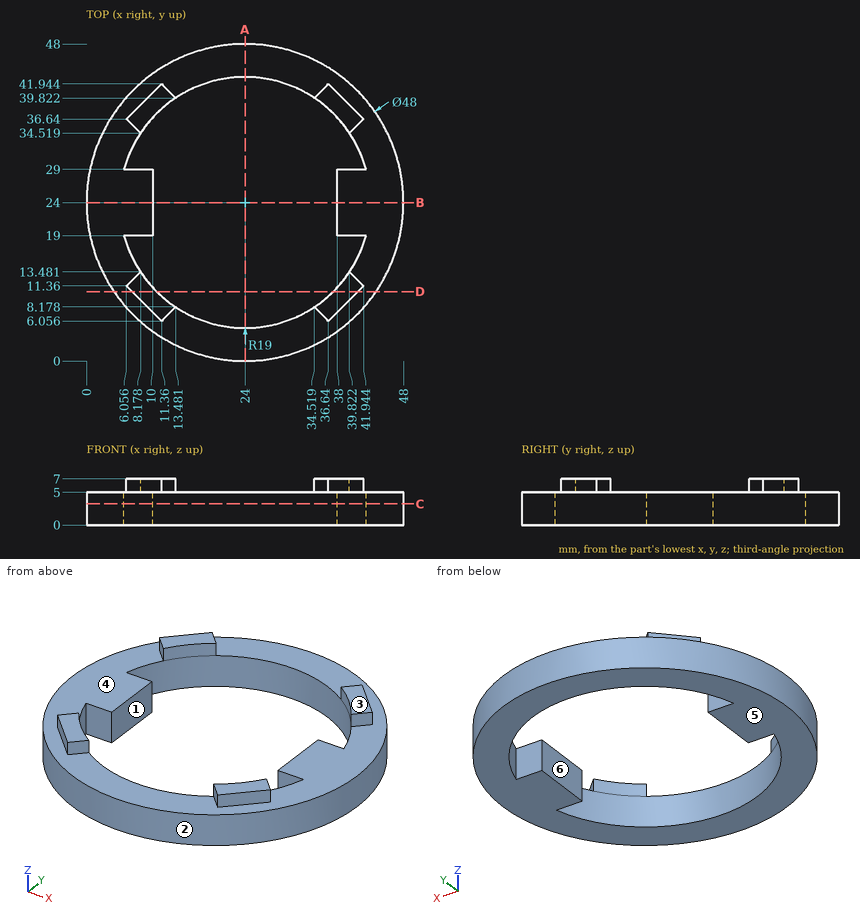
Part print with two shaded views. Sizes in mm from the minimum x, y, z corner. A direction names the side the tool comes from. Round coordinates to 2 decimals unless told otherwise and drop trailing zeros. Loops run counter-clockwise (first coordinate to the right, second up) from the corner with the lowest first, then second, coordinate; pieces in that order, holes last.
Item 1: Saw through at B-B (y = 24). List the corners of the cut face in (x, z).
Item 2: Which spindle directions (+Z, -Z, +X, -X, +Y, -Y) get a long thin tool onto all of the face, cutting with end or side? Do the marked faces 4, 5 and 6. Say none if no direction does.
Item 3: Two-plate mould, pull along Y, no slides. Class the marked faces 1, 2 and 3: released by +Y, released by -Y, zero draft, split by the parting line, or undercut.
Item 4: Saw through at D-D (y = 10.5). List the corners of the cut face in (x, z) (1 decimal).
Item 5: Saw through at A-A (x = 24). List the corners of the cut face in (y, z).
Item 6: Pin check, flat tips, straight feed: P1, Ø2, axis at y = 28, z = 3, coming from the -X side; P2, Ø4, axis at x = 33.5, z = 6, coming from the -Y side; P3, Ø3.5, axis at x = 39.5, z = 1.5, coming from the -Y side; P4, Ø6, axis at x = 17, y = 37.5, coming from the +Z side. Stop position of each tip, or through.
Item 7: Drill centre lines: line 1 along Y through (x, z) = (24.5, 3.25) (1 decimal); line 2 along Y through (x, z) = (7, 2.75) (1 decimal); line 3 along Z through (x, y) = (43, 16). Where is each one in solid material? Low to high.
Item 8: Saw through at C-C (z = 3.25). List the corners of the cut face in (x, y), then the cut area to 3 significant figures.
Worked answers:
1. outline: (0, 0) - (10, 0) - (10, 5) - (0, 5) - close; (38, 0) - (48, 0) - (48, 5) - (38, 5) - close
2. face 4: +Z
2. face 5: -Z, +X, -X, +Y, -Y
2. face 6: +Z, -Z
3. face 1: undercut
3. face 2: split by the parting line
3. face 3: zero draft
4. outline: (4.2, 0) - (10.6, 0) - (10.6, 7) - (6.9, 7) - (6.9, 5) - (4.2, 5) - close; (37.4, 0) - (43.8, 0) - (43.8, 5) - (41.1, 5) - (41.1, 7) - (37.4, 7) - close
5. outline: (0, 0) - (5, 0) - (5, 5) - (0, 5) - close; (43, 0) - (48, 0) - (48, 5) - (43, 5) - close
6. P1: stops at x = 0.19
6. P2: stops at y = 1.29
6. P3: stops at y = 4.33
6. P4: passes through
7. line 1: y = 0 to 5, 43 to 48
7. line 2: y = 7.1 to 15.5, 19 to 29, 32.5 to 40.9
7. line 3: z = 0 to 5
8. outline: circle Ø48 at (24, 24); hole (5.67, 19) arc R19 ccw to (42.33, 19) - (38, 19) - (38, 29) - (42.33, 29) arc R19 ccw to (5.67, 29) - (10, 29) - (10, 19) - close
8. area: 771 mm2
